Work out the finished part from the listing and answer in its coordinate system (mm). A direction names the side the tool comes from. Coordinates: 2 decimals unless noted, no trailing zeros. Write each loop counter-clockwise with the first axis right and the second up, starting at its lowest first coordinate (ties: lowest second). Pieces come first, ordered by that corner, then holes. Notation, with made-up numbers: (70, 50) - (112, 50) arc R8 ccw to (112, 59) - close; hole circle Ø7 at (19.25, -22). An arc over 180 degrees is marked (long way). Use a Markdown table: item, result. Add a question column.
(1) For a pull along Z with two mould halves and no side action, classify faces 1 (the face through (-565.91, 600.387, -17.587)), 2 (the face through (-449.565, 352.1, -19.786)), 3 (the face through (-630, 1265, 302)) as released by +Z, released by -Z, zero draft, split by the parting line, or undercut.
(2) The part is cut by section B-B, the plane z = -361. Give the vertices of the cut face in (x, y), then the cut area to 3 significant figures.
(3) The part is cut by section A-A, the plane z = 0. Give the vertices of the cut face in (x, y).
(4) Find the intervals of material crossed by line 1 (Y direction, x = -531.5, z = 0); line 2 (Z direction, x = 0, y = 274); line 3 (Z direction, x = 67, y = 647.5), in increasing order. Write a range as from..to.
(5) The part is cut by section C-C, the plane x = -528. Give the vertices of the cut face in (y, z), then the cut area to 3 significant figures.
(6) A tool of negligible diameter and unlimited length cuts with its end or side. For faces 4 (the face through (-302, 200, 265)), 5 (the face through (381.53, 352.1, -120.15)), 6 (the face through (-565.91, 550.435, -19.786)), from which of +Z, -Z, +X, -X, +Y, -Y can it reach the whole face along a straight path? Write none if from no direction.
(7) Given pin 1 Ø6 at (x, z) = (-40, 45.5) entering from +Y; pin 2 Ø1.5 at (x, y) = (-310.5, 489.5) entering from +Z; pin 3 Ø2 at (x, y) = (165.5, 627.5) entering from -Z, each flat-ended and moving along its own axis, determine where each tip first touches the part or whether it passes through.
from build123d import *

# Parameters (mm, degrees)
SKETCH1_R           = 450
SKETCH1_R_2         = 400
BOSS_EXTRUDE1_DEPTH = 750
SKETCH2_R           = 650
BOSS_EXTRUDE2_DEPTH = 100
SKETCH3_R           = 50
CUT_EXTRUDE1_DEPTH  = 1846.264208725
MOVE_FACE1_BY       = 750
SKETCH9_R           = 450
SKETCH9_R_2         = 400
SKETCH11_R          = 1265.740496662
CUT_EXTRUDE2_DEPTH  = 3153
MOVE_FACE2_BY       = 370
MOVE_FACE3_BY       = 200


with BuildPart() as part:
    # Sketch1 → Boss-Extrude1 (new, symmetric)
    with BuildSketch(Plane(origin=(0, 0, 0), x_dir=(1, 0, 0), z_dir=(0, 1, 0))):
        with Locations(Location((0, 0, 0), (0, 0, 270))):
            Circle(SKETCH1_R)
        with Locations(Location((0, 0, 0), (0, 0, 270))):
            Circle(SKETCH1_R_2, mode=Mode.SUBTRACT)
    extrude(amount=BOSS_EXTRUDE1_DEPTH, both=True)

    # Sketch2 → Boss-Extrude2 (add)
    with BuildSketch(Plane.XZ.offset(750)):
        with Locations(Location((0, 0, 0), (0, 0, 270))):
            Circle(SKETCH2_R)
    extrude(amount=BOSS_EXTRUDE2_DEPTH)

    # Sketch3 → Cut-Extrude1 (cut, through all)
    with BuildSketch(Plane.XZ.offset(850)):
        with Locations(Location((0, 550, 0), (0, 0, 270))):
            Circle(SKETCH3_R)
        with Locations(Location((550, 0, 0), (0, 0, 270))):
            Circle(SKETCH3_R)
        with Locations(Location((0, -550, 0), (0, 0, 270))):
            Circle(SKETCH3_R)
        with Locations(Location((-550, 0, 0), (0, 0, 270))):
            Circle(SKETCH3_R)
    extrude(amount=-CUT_EXTRUDE1_DEPTH, mode=Mode.SUBTRACT)

    # Move Face1: a face moved inward by 750.0
    extrude(part.faces().sort_by_distance((-225, 750, 360))[0], amount=MOVE_FACE1_BY, dir=(0, -1, 0), mode=Mode.SUBTRACT)

    # Sweep1: sweep along a path in Sketch8
    with BuildLine(Plane.XY) as sweep1_path:
        Line((0, 0), (0, 500))
        ThreePointArc((0, 500), (-146.446609407, 853.553390593), (-500, 1000))
        Line((-500, 1000), (-1000, 1000))
    # Sketch9 → Sweep1 (sweep)
    with BuildSketch(Plane(origin=(0, 0, 0), x_dir=(1, 0, 0), z_dir=(0, 1, 0))):
        Circle(SKETCH9_R)
        Circle(SKETCH9_R_2, mode=Mode.SUBTRACT)
    sweep(path=sweep1_path.line)

    # Sketch11 → Cut-Extrude2 (cut)
    with BuildSketch(Plane(origin=(0, 0, 0), x_dir=(1, 0, 0), z_dir=(0, 1, 0))):
        with Locations((-18.825691705, 0)):
            Circle(SKETCH11_R)
    extrude(amount=-CUT_EXTRUDE2_DEPTH, mode=Mode.SUBTRACT)

    # Move Face2: a face moved inward by 370.0
    extrude(part.faces().sort_by_distance((-1000, 1360, 225))[0], amount=MOVE_FACE2_BY, dir=(1, 0, 0), mode=Mode.SUBTRACT)

    # Move Face3: a face moved inward by 200.0
    extrude(part.faces().sort_by_distance((-225, 0, 360))[0], amount=MOVE_FACE3_BY, dir=(0, 1, 0), mode=Mode.SUBTRACT)


solid = part.part
Model answer:
| question | item | result |
|---|---|---|
| 1 | face 1 | undercut |
| 1 | face 2 | split by the parting line |
| 1 | face 3 | zero draft |
| 2 | outline | (-630, 731.34) - (-500, 731.34) arc R231.34 cw to (-268.66, 500) - (-268.66, 200) - (-172.28, 200) - (-172.28, 500) arc R327.72 ccw to (-500, 827.72) - (-630, 827.72) - close; (-630, 1172.28) - (-500, 1172.28) arc R672.28 cw to (172.28, 500) - (172.28, 200) - (268.66, 200) - (268.66, 500) arc R768.66 ccw to (-500, 1268.66) - (-630, 1268.66) - close |
| 2 | area | 234,000 mm^2 |
| 3 | outline | (-630, 550) - (-500, 550) arc R50 cw to (-450, 500) - (-450, 200) - (-400, 200) - (-400, 500) arc R100 ccw to (-500, 600) - (-630, 600) - close; (-630, 1400) - (-500, 1400) arc R900 cw to (400, 500) - (400, 200) - (450, 200) - (450, 500) arc R950 ccw to (-500, 1450) - (-630, 1450) - close |
| 4 | line 1 | 550..600, 1400..1450 |
| 4 | line 2 | -450..-400, 400..450 |
| 4 | line 3 | -441.73..-390.67, 390.67..441.73 |
| 5 | outline | circle Ø900 at (1000, 0); hole circle Ø800 at (1000, 0) |
| 5 | area | 134,000 mm^2 |
| 6 | face 4 | +Z, -Z, +X, -X, -Y |
| 6 | face 5 | -Y |
| 6 | face 6 | -X |
| 7 | pin 1 | y = 1330.26 |
| 7 | pin 2 | z = 326.43 |
| 7 | pin 3 | z = -413.9 |
